Geometry check sheet. Reference: the model listing, model coordinates, mm. A direction names the side the tool comes from. Give positions to 0.01 mm unless a question says otherwise; leave off trailing zeros. Loops run counter-clockwise (first coordinate to the right, second up) from the corner with the lowest first, then second, coordinate; pieces in that order, holes last.
1. Cross-section at D-D, the plane z = 21.5. Record the cut outline in (x, y), plus the area to 3 significant figures.
2. Cross-section at A-A, the plane y = 0. Record the cut outline in (x, z).
3. Go/stop test with flat-tipped pins: pin 1 Ø7 at (x, z) = (18, 11.75) entering from -Y; pin 2 Ø12 at (y, z) = (-6.5, 9) entering from +X; pin 3 Ø4 at (x, z) = (21, 10.5) entering from -Y; pin 4 Ø2.5 at (x, z) = (-18, 11.75) entering from -Y. Record where each tip stops, or that it passes through.
4. Cross-section at B-B, the plane z = 11.75. State how many separate pieces and enclosed holes the cut face has, plus the area to 3 significant figures.
5. Tool access check on faces 1 (the flat face through (-24, -2, 12)), 2 (the flat face through (24, -2, 12)), 3 (the flat face through (-8, 18, 12)). Record the directions out of +Z, -Z, +X, -X, +Y, -Y that give a thin tool (end or side, any length) a straight path to the whole face; none if there is none.
6. Cross-section at C-C, the plane x = 0. Record the cut outline in (y, z), plus the area to 3 significant figures.
7. Release check for a two-part mould opening along Z. For faces 4 (the flat face through (0, 9, 23.5)), 5 (the cylindrical face through (15.9, 2.75, 11.28)), 6 (the flat face through (8, 18, 12)) record: +Z half, -Z half, draft (parallel to the pull), parting line (faces both ways), or undercut.
8. Material ranges on L1, parallel to X at y = 9, z = 11.75; L2, parallel to Y at x = 0, z = 13.25; L3, parallel to X at y = -2, z = 13.5, recorded low to high.
from build123d import *

# Parameters (mm, degrees)
SKETCH_1_R          = 8
EXTRUDE_1_DEPTH     = 23.5
SKETCH_2_R          = 2.15
CUT_EXTRUDE_1_DEPTH = 52.570340313


with BuildPart() as part:
    # 草图1 → 凸台-拉伸1 (new body)
    with BuildSketch(Plane.XY):
        Polygon((-10.25, -19.5), (10.25, -19.5), (16.25, -13.5), (24, -13.5), (24, 9), (25, 10), (25, 18.5), (24.5, 19), (13.5, 19), (12.5, 18), (4, 18), (3, 19), (-3, 19), (-4, 18), (-12.5, 18), (-13.5, 19), (-24.5, 19), (-25, 18.5), (-25, 10), (-24, 9), (-24, -13.5), (-16.25, -13.5), align=None)
        Circle(SKETCH_1_R, mode=Mode.SUBTRACT)
    extrude(amount=EXTRUDE_1_DEPTH)

    # 草图2 → 切除-拉伸1 (cut, through all)
    with BuildSketch(Plane(origin=(0, 19, 0), x_dir=(1, 0, 0), z_dir=(0, 1, 0))):
        with Locations(Location((-18, -11.75, 0), (0, 0, 270))):
            Circle(SKETCH_2_R)
        with Locations(Location((18, -11.75, 0), (0, 0, 270))):
            Circle(SKETCH_2_R)
    extrude(amount=-CUT_EXTRUDE_1_DEPTH, mode=Mode.SUBTRACT)


solid = part.part
Result:
1. outline: (-25, 10) - (-24, 9) - (-24, -13.5) - (-16.25, -13.5) - (-10.25, -19.5) - (10.25, -19.5) - (16.25, -13.5) - (24, -13.5) - (24, 9) - (25, 10) - (25, 18.5) - (24.5, 19) - (13.5, 19) - (12.5, 18) - (4, 18) - (3, 19) - (-3, 19) - (-4, 18) - (-12.5, 18) - (-13.5, 19) - (-24.5, 19) - (-25, 18.5) - close; hole circle Ø16 at (0, 0)
1. area: 1,520 mm2
2. outline: (-24, 0) - (-8, 0) - (-8, 23.5) - (-24, 23.5) - close; (8, 0) - (24, 0) - (24, 23.5) - (8, 23.5) - close; hole circle Ø4.3 at (-18, 11.75); hole circle Ø4.3 at (18, 11.75)
3. pin 1: stops at y = -15.25
3. pin 2: stops at x = 24
3. pin 3: stops at y = -13.5
3. pin 4: passes through
4. separate pieces: 3
4. enclosed holes: 1
4. area: 1,240 mm2
5. face 1: +Z, -Z, -X, -Y
5. face 2: +Z, -Z, +X, -Y
5. face 3: +Z, -Z, +Y
6. outline: (-19.5, 0) - (-8, 0) - (-8, 23.5) - (-19.5, 23.5) - close; (8, 0) - (19, 0) - (19, 23.5) - (8, 23.5) - close
6. area: 529 mm2
7. face 4: +Z half
7. face 5: undercut
7. face 6: draft
8. L1: x = -24 to -20.15, -15.85 to 15.85, 20.15 to 24
8. L2: y = -19.5 to -8, 8 to 19
8. L3: x = -24 to -19.25, -16.75 to -7.75, 7.75 to 16.75, 19.25 to 24
